from build123d import *

# Parameters (mm, degrees)
SKETCH1_R               = 15
LINEAR_AUSTRAGEN1_DEPTH = 8


with BuildPart() as part:
    # Sketch1 → Linear austragen1 (new body)
    with BuildSketch(Plane.XY):
        with BuildLine():
            Line((-46.490516198, 101.722073941), (-16.145123023, 345.436482626))
            ThreePointArc((-16.145123023, 345.436482626), (-14.553663061, 348.512142372), (-11.345515054, 349.816064937))
            ThreePointArc((-11.345515054, 349.816064937), (24.425679263, 349.146654277), (59.941644882, 344.828941954))
            ThreePointArc((59.941644882, 344.828941954), (63.893687736, 341.27385411), (62.410890197, 336.16909126))
            Line((62.410890197, 336.16909126), (27.68409004, 305.238604713))
            ThreePointArc((27.68409004, 305.238604713), (23.620398385, 299.316491146), (22.775693358, 292.184065725))
            Line((22.775693358, 292.184065725), (46.490516198, 101.722073941))
            ThreePointArc((46.490516198, 101.722073941), (58.778525229, 80.901699437), (82.37708169, 75.648957927))
            Line((82.37708169, 75.648957927), (323.540500377, 122.100668066))
            ThreePointArc((323.540500377, 122.100668066), (326.957414795, 121.537530829), (329.188891102, 118.889334994))
            ThreePointArc((329.188891102, 118.889334994), (339.606150684, 84.662048273), (346.474799191, 49.550111254))
            ThreePointArc((346.474799191, 49.550111254), (344.314958136, 44.692912585), (339.001830525, 44.525678373))
            Line((339.001830525, 44.525678373), (298.854018333, 67.994781966))
            ThreePointArc((298.854018333, 67.994781966), (291.966003854, 70.02954866), (284.921635971, 68.628870213))
            Line((284.921635971, 68.628870213), (111.109800855, -12.781258825))
            ThreePointArc((111.109800855, -12.781258825), (95.10565163, -30.901699437), (97.402352577, -54.968446729))
            Line((97.402352577, -54.968446729), (216.104148993, -269.974119712))
            ThreePointArc((216.104148993, -269.974119712), (216.624458278, -273.397817411), (214.795438474, -276.338415011))
            ThreePointArc((214.795438474, -276.338415011), (185.462464648, -296.822630887), (154.191557264, -314.205289052))
            ThreePointArc((154.191557264, -314.205289052), (148.904659228, -313.652115076), (147.103763315, -308.650708653))
            Line((147.103763315, -308.650708653), (157.017850965, -263.215518401))
            ThreePointArc((157.017850965, -263.215518401), (156.824515556, -256.035849857), (153.315561803, -249.769091324))
            Line((153.315561803, -249.769091324), (22.179117214, -109.621326314))
            ThreePointArc((22.179117214, -109.621326314), (0, -100), (-22.179117214, -109.621326314))
            Line((-22.179117214, -109.621326314), (-189.980791189, -288.953850131))
            ThreePointArc((-189.980791189, -288.953850131), (-193.076136784, -290.506674439), (-196.438009496, -289.675867868))
            ThreePointArc((-196.438009496, -289.675867868), (-224.984043894, -268.108522791), (-251.179176024, -243.739659333))
            ThreePointArc((-251.179176024, -243.739659333), (-252.28681765, -238.540580345), (-248.086704923, -235.282306972))
            Line((-248.086704923, -235.282306972), (-201.811649597, -230.670918704))
            ThreePointArc((-201.811649597, -230.670918704), (-195.043122971, -228.26840621), (-190.167407773, -222.99465799))
            Line((-190.167407773, -222.99465799), (-97.402352577, -54.968446729))
            ThreePointArc((-97.402352577, -54.968446729), (-95.10565163, -30.901699437), (-111.109800855, -12.781258825))
            Line((-111.109800855, -12.781258825), (-333.518735158, 91.390819151))
            ThreePointArc((-333.518735158, 91.390819151), (-335.952073227, 93.854818649), (-336.200805025, 97.308882948))
            ThreePointArc((-336.200805025, 97.308882948), (-324.510250701, 131.122451129), (-309.428825313, 163.565895178))
            ThreePointArc((-309.428825313, 163.565895178), (-304.826487449, 166.225928727), (-300.429779115, 163.238245993))
            Line((-300.429779115, 163.238245993), (-281.744309741, 120.653050426))
            ThreePointArc((-281.744309741, 120.653050426), (-277.367794824, 114.958216262), (-270.845483359, 111.950813376))
            Line((-270.845483359, 111.950813376), (-82.37708169, 75.648957927))
            ThreePointArc((-82.37708169, 75.648957927), (-58.778525229, 80.901699437), (-46.490516198, 101.722073941))
        make_face()
        Circle(SKETCH1_R, mode=Mode.SUBTRACT)
    extrude(amount=LINEAR_AUSTRAGEN1_DEPTH)


solid = part.part
Geometry: final body of the model. Coordinates: model frame, mm. A direction names the side the tool comes from. Coordinates: 2 decimals unless noted, no trailing zeros. Loops run counter-clockwise (first coordinate to the right, second up) from the corner with the lowest first, then second, coordinate; pieces in that order, holes last. Notation, with made-up numbers: (41, 75.5) - (61, 75.5) arc R19 cw to (61, 96.5) - close; hole circle Ø10 at (-27.5, 38.25). An arc over 180 degrees is marked (long way). Put each result on its own line as item: value. Start each with the question number.
Q1. Line query: line 1 (Y direction, x = 0, z = 5.25); line 2 (X direction, y = -191, z = 6.5); line 3 (Y direction, x = 202, z = 3.5). Output: solid intervals per line, ascending.
Q2. Cut plane D-D, the plane y = -87. Return loops of the section in (x, z).
Q3. Cut plane B-B, the plane y = 143. Return loops of the section in (x, z), and give its area (3 significant figures).
Q4. Cut plane A-A, the plane x = 0. Return loops of the section in (y, z), and give its area (3 significant figures).
Q5. Pull-direction query (Y, two-part tool) for faces 6 (the flat face through (-19, -5, 8)), 7 (the flat face through (155.922, -160.966, 3.944)), 8 (the flat face through (45.29, 320.92, 3.94)), 9 (the flat face through (-177.931, 94.054, 3.944)); classes: released by +Y, released by -Y, zero draft, split by the parting line, or undercut.
Q6. Set-up query: faces 1 (the flat face through (-220.757, 38.576, 3.944)), 2 (the flat face through (-291.2, 142.2, 3.9)), 3 (the cylindrical face through (95.215, -30.571, 3.944)), 4 (the cylindrical face through (58.498, 81.108, 3.944)), 5 (the flat face through (-104.905, -198.032, 3.944)). Return all of +Z, -Z, +X, -X, +Y, -Y with unobstructed straight access to the full face (end or side cutting, diameter ignored); none if empty.
Q7. Cut plane C-C, the plane y = 282. Return loops of the section in (x, z).
Q8. Pin query (flat end, axial travel): pin 1 Ø2 at (x, z) = (194.5, 2) entering from -Y; pin 2 Ø18 at (x, y) = (0, 0) entering from +Z; pin 3 Ø3 at (x, y) = (182, -208.5) entering from -Z; pin 4 Ø1 at (x, z) = (208, 2) entering from -Y. Return the tip coordinate at first contact, or that it passes through.
Filled sheet:
1. line 1: -100 to -15, 15 to 350
1. line 2: -172.5 to -98.33, 98.33 to 172.5
1. line 3: -285.83 to -244.43, 29.79 to 98.69
2. outline: (-115.09, 0) - (115.09, 0) - (115.09, 8) - (-115.09, 8) - close
3. outline: (-319.45, 0) - (-291.55, 0) - (-291.55, 8) - (-319.45, 8) - close; (-41.35, 0) - (41.35, 0) - (41.35, 8) - (-41.35, 8) - close
3. area: 885 mm²
4. outline: (-100, 0) - (-15, 0) - (-15, 8) - (-100, 8) - close; (15, 0) - (350, 0) - (350, 8) - (15, 8) - close
4. area: 3,360 mm²
5. face 6: zero draft
5. face 7: undercut
5. face 8: undercut
5. face 9: released by +Y
6. face 1: +Z, -Z, -X
6. face 2: +Z, -Z, +Y
6. face 3: +Z, -Z, +X
6. face 4: +Z, -Z
6. face 5: +Z, -Z, -Y
7. outline: (-24.04, 0) - (24.04, 0) - (24.04, 8) - (-24.04, 8) - close
8. pin 1: y = -291.65
8. pin 2: through
8. pin 3: z = 0
8. pin 4: y = -281.86
